Read the model definition and answer for the solid it produces. Units are mm, in the model's axes. Face numbers are marked on the shaded views. A direction names the side the tool comes from. Coordinates: 2 decimals unless noted, no trailing zeros. Order: outer loops, then holes, each group sorted by start corner. A loop starts at its lowest first (then second) coordinate and runs counter-clockwise, first axis right, second up. Notation, with made-up numbers: (72.5, 74) -> (118.5, 74) arc R17 cw to (118.5, 104) -> close; hole circle Ø9 at (74.25, -16.75). An arc over 180 degrees is marked (long way). Answer as a JSON object with one key per item and string values. Group by question number.
1) Determine the mould class of the marked faces 1, 2 and 3 for opening direction X: released by +X, released by -X, zero draft, split by the parting line, or undercut.
2) Consider L1, parallel to X at y = -0.5, z = 2; L2, parallel to Y at x = 0, z = 2.2; L3, parallel to Y at x = 0, z = 3.7. Determine where each line is inside the solid, lowest interval first.
3) Given pin 1 (3 mm diameter, centred on x = 2.5, z = 5.5, fed in from +Y); pin 2 (12 mm diameter, centred on x = 18.5, y = -7.5, fed in from +Z); pin 3 (3 mm diameter, centred on x = -15.5, z = 2.5, fed in from +Y); pin 4 (3 mm diameter, centred on x = 10.5, z = 4, fed in from -Y), each flat-ended and moving along its own axis, determine where each tip first touches the part or whether it passes through.
4) A tool of negligible diameter and unlimited length cuts with its end or side. For the marked faces 4 and 5, from which of +Z, -Z, +X, -X, +Y, -Y can it reach the whole face along a straight path? Write none if from no direction.
5) Section A-A on y = 0 is taken. Determine the outline of the cut face in (x, z), and give its area (3 significant figures).
6) Section C-C on z = 2 is taken. Determine the outline of the cut face in (x, y), and give its area (3 significant figures).
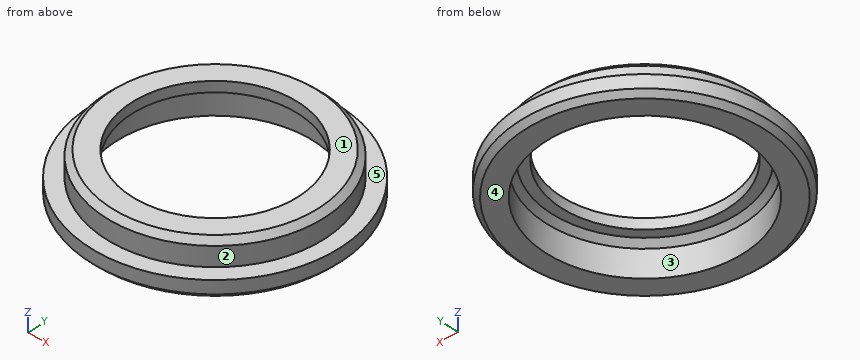
from build123d import *

# Parameters (mm, degrees)
SKETCH_1_R      = 24
SKETCH_1_R_2    = 19
EXTRUDE_1_DEPTH = 3.5
SKETCH_2_R      = 21
SKETCH_2_R_2    = 19
EXTRUDE_2_DEPTH = 2.8
SKETCH_3_R      = 21
SKETCH_3_R_2    = 16
EXTRUDE_3_DEPTH = 2
CHAMFER_1_SIZE  = 1.1
CHAMFER_2_SIZE  = 1


with BuildPart() as part:
    # 草图1 → 凸台-拉伸1 (new body)
    with BuildSketch(Plane.XY):
        Circle(SKETCH_1_R)
        Circle(SKETCH_1_R_2, mode=Mode.SUBTRACT)
    extrude(amount=EXTRUDE_1_DEPTH)

    # 草图2 → 凸台-拉伸2 (add)
    with BuildSketch(Plane.XY.offset(3.5)):
        Circle(SKETCH_2_R)
        Circle(SKETCH_2_R_2, mode=Mode.SUBTRACT)
    extrude(amount=EXTRUDE_2_DEPTH)

    # 草图3 → 凸台-拉伸3 (add)
    with BuildSketch(Plane.XY.offset(6.3)):
        Circle(SKETCH_3_R)
        Circle(SKETCH_3_R_2, mode=Mode.SUBTRACT)
    extrude(amount=EXTRUDE_3_DEPTH)

    # 倒角1
    chamfer_1_edges = [part.edges().sort_by_distance(p)[0] for p in [
        (-21, 0, 8.3),
        (-19, 0, 6.3),
    ]]
    chamfer(chamfer_1_edges, length=CHAMFER_1_SIZE)

    # 倒角2
    chamfer_2_edges = [part.edges().sort_by_distance(p)[0] for p in [
        (-24, 0, 0),
    ]]
    chamfer(chamfer_2_edges, length=CHAMFER_2_SIZE)


solid = part.part
Worked answers:
{
 "1": {"face 1": "zero draft", "face 2": "split by the parting line", "face 3": "undercut"},
 "2": {"L1": "x = -23.99 to -18.99, 18.99 to 23.99", "L2": "y = -24 to -19, 19 to 24", "L3": "y = -21 to -19, 19 to 21"},
 "3": {"pin 1": "stops at y = 20.98", "pin 2": "stops at z = 8.3", "pin 3": "stops at y = 19.49", "pin 4": "stops at y = -22.21"},
 "4": {"face 4": "-Z, +X, -X, +Y, -Y", "face 5": "+Z"},
 "5": {"outline": "(-24, 1) -> (-23, 0) -> (-19, 0) -> (-19, 5.2) -> (-17.9, 6.3) -> (-16, 6.3) -> (-16, 8.3) -> (-19.9, 8.3) -> (-21, 7.2) -> (-21, 3.5) -> (-24, 3.5) -> close; (16, 6.3) -> (17.9, 6.3) -> (19, 5.2) -> (19, 0) -> (23, 0) -> (24, 1) -> (24, 3.5) -> (21, 3.5) -> (21, 7.2) -> (19.9, 8.3) -> (16, 8.3) -> close", "area": "65.2 mm²"},
 "6": {"outline": "circle Ø48 at (0, 0); hole circle Ø38 at (0, 0)", "area": "675 mm²"}
}
